Design review of the part built by this model. Coordinates are the model's own, in mm. A direction names the side the tool comes from. Coordinates: 2 decimals unless noted, no trailing zeros. Order: outer loops, then holes, each group sorted by start corner. A loop starts at its lowest first (then second) coordinate and runs counter-clockwise, first axis right, second up. Notation, with made-up numbers: (-11.5, 16.5) -> (35.5, 16.5) arc R26 ccw to (35.5, 42.5) -> close; hole circle Ø1 at (53, 71.25). An arc over 180 degrees is marked (long way). Write item = value, one per line.
```python
from build123d import *

# Parameters (mm, degrees)
BOSS_EXTRUDE1_DEPTH            = 202
CUT_EXTRUDE1_START             = -16
CUT_EXTRUDE1_DEPTH             = 16
CUT_EXTRUDE2_DEPTH             = 18
CUT_EXTRUDE3_DEPTH             = 30
BOSS_EXTRUDE2_START            = 2
BOSS_EXTRUDE2_DEPTH            = 2
BOSS_EXTRUDE3_DEPTH            = 6
BOSS_EXTRUDE4_DEPTH            = 30
F_16_0_16_DIAMETER_HOLE1_D     = 16
F_16_0_16_DIAMETER_HOLE1_DEPTH = 20
F_12_0_12_DIAMETER_HOLE1_D     = 12
F_12_0_12_DIAMETER_HOLE1_DEPTH = 34


with BuildPart() as part:
    # Sketch1 → Boss-Extrude1 (new body)
    with BuildSketch(Plane(origin=(0, 0, -358.692981355), x_dir=(-1, 0, 0), z_dir=(0, 0, -1))):
        with BuildLine():
            Line((-707.84521865, 246.743963655), (-726.230642584, 246.743963655))
            Line((-726.230642584, 246.743963655), (-726.230642584, 234.743963655))
            Line((-726.230642584, 234.743963655), (-316.230642584, 234.743963655))
            Line((-316.230642584, 234.743963655), (-316.230642584, 246.743963655))
            Line((-316.230642584, 246.743963655), (-334.616066519, 246.743963655))
            ThreePointArc((-334.616066519, 246.743963655), (-521.230642584, 421.743963655), (-707.84521865, 246.743963655))
        make_face()
    extrude(amount=-BOSS_EXTRUDE1_DEPTH)

    # Sketch2 → Cut-Extrude1 (cut)
    with BuildSketch(Plane.XY.offset(-156.692981355).offset(CUT_EXTRUDE1_START)):
        with BuildLine():
            Line((640.629135037, 246.743963655), (707.84521865, 246.743963655))
            ThreePointArc((707.84521865, 246.743963655), (521.230642584, 421.743963655), (334.616066519, 246.743963655))
            Line((334.616066519, 246.743963655), (401.832150132, 246.743963655))
            ThreePointArc((401.832150132, 246.743963655), (521.230642584, 354.743963655), (640.629135037, 246.743963655))
        make_face()
    extrude(amount=CUT_EXTRUDE1_DEPTH, mode=Mode.SUBTRACT)

    # Sketch3 → Cut-Extrude2 (cut)
    with BuildSketch(Plane(origin=(0, 0, -358.692981355), x_dir=(-1, 0, 0), z_dir=(0, 0, -1))):
        with BuildLine():
            Line((-371.711413052, 246.743963655), (-334.616066519, 246.743963655))
            ThreePointArc((-334.616066519, 246.743963655), (-521.230642584, 421.743963654), (-707.84521865, 246.743963655))
            Line((-707.84521865, 246.743963655), (-670.749872117, 246.743963655))
            ThreePointArc((-670.749872117, 246.743963655), (-521.230642584, 384.743963654), (-371.711413052, 246.743963655))
        make_face()
    extrude(amount=-CUT_EXTRUDE2_DEPTH, mode=Mode.SUBTRACT)

    # Sketch4 → Cut-Extrude3 (cut)
    with BuildSketch(Plane(origin=(0, 0, -340.692981355), x_dir=(-1, 0, 0), z_dir=(0, 0, -1))):
        with BuildLine():
            Line((-707.84521865, 246.743963655), (-334.616066519, 246.743963655))
            ThreePointArc((-334.616066519, 246.743963655), (-521.230642584, 421.743963655), (-707.84521865, 246.743963655))
        make_face()
    extrude(amount=-CUT_EXTRUDE3_DEPTH, mode=Mode.SUBTRACT)

    # Sketch5 → Boss-Extrude2 (add)
    with BuildSketch(Plane(origin=(0, 0, -358.692981355), x_dir=(-1, 0, 0), z_dir=(0, 0, -1)).offset(BOSS_EXTRUDE2_START)):
        with BuildLine():
            Line((-371.230642584, 234.743963655), (-671.230642584, 234.743963655))
            ThreePointArc((-671.230642584, 234.743963655), (-521.230642584, 384.743963655), (-371.230642584, 234.743963655))
        make_face()
    extrude(amount=-BOSS_EXTRUDE2_DEPTH)

    # Sketch6 → Boss-Extrude3 (add)
    with BuildSketch(Plane.XY.offset(-156.692981355)):
        with BuildLine():
            Line((641.230642584, 234.743963655), (401.230642584, 234.743963655))
            ThreePointArc((401.230642584, 234.743963655), (521.230642584, 354.743963655), (641.230642584, 234.743963655))
        make_face()
    extrude(amount=BOSS_EXTRUDE3_DEPTH)

    # Sketch7 → Boss-Extrude4 (add)
    with BuildSketch(Plane.XY.offset(-340.692981355)):
        with BuildLine():
            Line((619.500678709, 246.743963655), (422.960606459, 246.743963655))
            ThreePointArc((422.960606459, 246.743963655), (521.230642584, 333.743963655), (619.500678709, 246.743963655))
        make_face()
    extrude(amount=BOSS_EXTRUDE4_DEPTH)

    # Sketch8 → Cut-Revolve1 (revolve, cut)
    with BuildSketch(Plane(origin=(0, 234.743963655, 0), x_dir=(1, 0, 0), z_dir=(0, 1, 0))):
        Polygon((606.230642584, 360.692981355), (521.230642584, 360.692981355), (521.230642584, 150.692981355), (606.230642584, 150.692981355), (606.230642584, 184.692981355), (696.230642584, 184.692981355), (696.230642584, 298.692981355), (606.230642584, 298.692981355), align=None)
    revolve(axis=Axis((521.230642584, 234.743963655, -360.692981355), (0, 0, 1)), mode=Mode.SUBTRACT)

    # Ø16.0 (16) diameter hole1
    with Locations(Plane.XY.offset(-340.692981355)):
        with Locations((421.637721149, 292.243963655), (620.82356402, 292.243963655)):
            Hole(F_16_0_16_DIAMETER_HOLE1_D / 2, depth=F_16_0_16_DIAMETER_HOLE1_DEPTH)

    # Ø12.0 (12) diameter hole1
    with Locations(Plane.XY.offset(-150.692981355)):
        with Locations((521.230642584, 337.243963655), (432.463038696, 285.993963655), (609.998246472, 285.993963655)):
            Hole(F_12_0_12_DIAMETER_HOLE1_D / 2, depth=F_12_0_12_DIAMETER_HOLE1_DEPTH)


solid = part.part
```
(1) For L1, parallel to Z at x = 470, y = 342.5; L2, parallel to Z at x = 528.5, y = 384; L3, parallel to Z at x = 483, y = 312, list the stretches that pass through material, from the lowest coordinate up.
Report:
L1 = -360.69 to -340.69, -310.69 to -298.69, -184.69 to -150.69
L2 = -360.69 to -340.69, -310.69 to -298.69, -184.69 to -172.69
L3 = -360.69 to -298.69, -184.69 to -150.69
(2) Insertion check: pin 1 (9.5 mm diameter, centred on x = 350.5, y = 238.5, fed in from +Z); pin 2 (3 mm diameter, centred on x = 604.5, z = -210.5, fed in from +Y); pin 3 (13 mm diameter, centred on x = 709, y = 243, fed in from -Z). Each pin has a flat end and moves straight along its axis. Give the tip position at first contact, or say it passes through.
Report:
pin_1 = -156.69
pin_2 = 402.92
pin_3 = -358.69
(3) We need section D-D (z = -177.5). Write out the cut boundary in (x, y), and give its area (3 significant figures).
Report:
outline = (316.23, 234.74) -> (436.23, 234.74) arc R85 cw to (606.23, 234.74) -> (726.23, 234.74) -> (726.23, 246.74) -> (707.85, 246.74) arc R187 ccw to (334.62, 246.74) -> (316.23, 246.74) -> close; hole circle Ø12 at (432.46, 285.99); hole circle Ø12 at (521.23, 337.24); hole circle Ø12 at (610, 285.99)
area = 43,700 mm²
(4) The part is to be moulded in two halves that separate along X. For faces 5 (the cylindrical face through (517.287, 421.702, -242.659)), 6 (the cylindrical face through (525.1, 409.7, -242.5)), 7 (the flat face through (519, 355, -172.693)), say which applies: released by +X, released by -X, zero draft, split by the parting line, or undercut.
Report:
face_5 = split by the parting line
face_6 = undercut
face_7 = zero draft
(5) We need section A-A (z = -214). Write out the cut boundary in (x, y).
Report:
outline = (316.23, 234.74) -> (346.23, 234.74) arc R175 cw to (696.23, 234.74) -> (726.23, 234.74) -> (726.23, 246.74) -> (707.85, 246.74) arc R187 ccw to (334.62, 246.74) -> (316.23, 246.74) -> close
(6) We need section C-C (x = 496). Write out the cut boundary in (y, z), and give its area (3 significant figures).
Report:
outline = (315.91, -360.69) -> (382.61, -360.69) -> (382.61, -340.69) -> (330.47, -340.69) -> (330.47, -310.69) -> (420.03, -310.69) -> (420.03, -172.69) -> (352.06, -172.69) -> (352.06, -150.69) -> (315.91, -150.69) -> (315.91, -184.69) -> (407.92, -184.69) -> (407.92, -298.69) -> (315.91, -298.69) -> close
area = 6,450 mm²
(7) We need section B-B (y = 326.5). Write out the cut boundary in (x, z).
Report:
outline = (358.29, -310.69) -> (484.06, -310.69) -> (484.06, -340.69) -> (402.57, -340.69) -> (402.57, -360.69) -> (639.89, -360.69) -> (639.89, -340.69) -> (558.4, -340.69) -> (558.4, -310.69) -> (684.17, -310.69) -> (684.17, -172.69) -> (598.57, -172.69) -> (598.57, -150.69) -> (443.89, -150.69) -> (443.89, -172.69) -> (358.29, -172.69) -> close; hole (372.21, -298.69) -> (670.25, -298.69) -> (670.25, -184.69) -> (372.21, -184.69) -> close
(8) For faces 1 (the flat face through (360, 241, -156.693)), 2 (the flat face through (344, 241, -358.693)), 3 (the cylindrical face through (614.76, 282.343, -167.931)), 4 (the flat face through (333, 246.744, -259)), list the 3-axis set-ups (+Z, -Z, +X, -X, +Y, -Y) from which the entire face can be reached by the end or side of a thin tool; tool diameter is ignored.
Report:
face_1 = +Z, -X, +Y, -Y
face_2 = -Z, -X, +Y, -Y
face_3 = +Z
face_4 = -X, +Y
